Source: three-view drawing plus pictorial views. Frame: mm from the lowest corner of the part. Round coordinates to 2 decimals unless told otherwise and drop trailing zeros. Loops run counter-clockwise (first coordinate to the right, second up) from the corner with the lowest first, then second, coordinate; pieces in that order, holes last. Notation, with made-up numbers: (-39.75, 6.5) -> (16.25, 6.5) arc R14 cw to (16.25, 26.5) -> close; hole circle Ø9 at (-4.5, 33). An arc over 180 degrees is marked (long way). Answer in a Markdown table with one row per item. Add a question column.
Q1. Section C-C, the plane x = 54. Output: boundary loops of the cut face in (y, z), and give its area (3 significant figures).
Q2. Section D-D, the plane z = 42. Output: boundary loops of the cut face in (x, y), and give its area (3 significant figures).
Q3. Ray query, L1, parallel to Y at x = 71, z = 27; L2, parallel to X at y = 30, z = 50.5; L3, parallel to Z at x = 57, y = 38.5. Return the intervals inside material, ascending. Write a range as from..to.
Q4. Mould query, pull axis Z, two halves, no side actions, for the marked faces 1, 2 and 3. Classes: pulls with the +Z half, pulls with the -Z half, needs draft (parallel to the pull), parting line crosses it, or undercut.
Q5. Section A-A, the plane z = 27. Output: boundary loops of the cut face in (x, y), and give its area (3 significant figures).
Q6. Pin query (flat end, axial travel): pin 1 (3 mm diameter, centred on y = 48, z = 45.5, fed in from +X); pin 2 (3 mm diameter, centred on x = 49.5, y = 45.5, fed in from -Z); pin 3 (1 mm diameter, centred on x = 88.5, y = 17.5, fed in from +Z). Return the tip coordinate at first contact, or that it passes through.
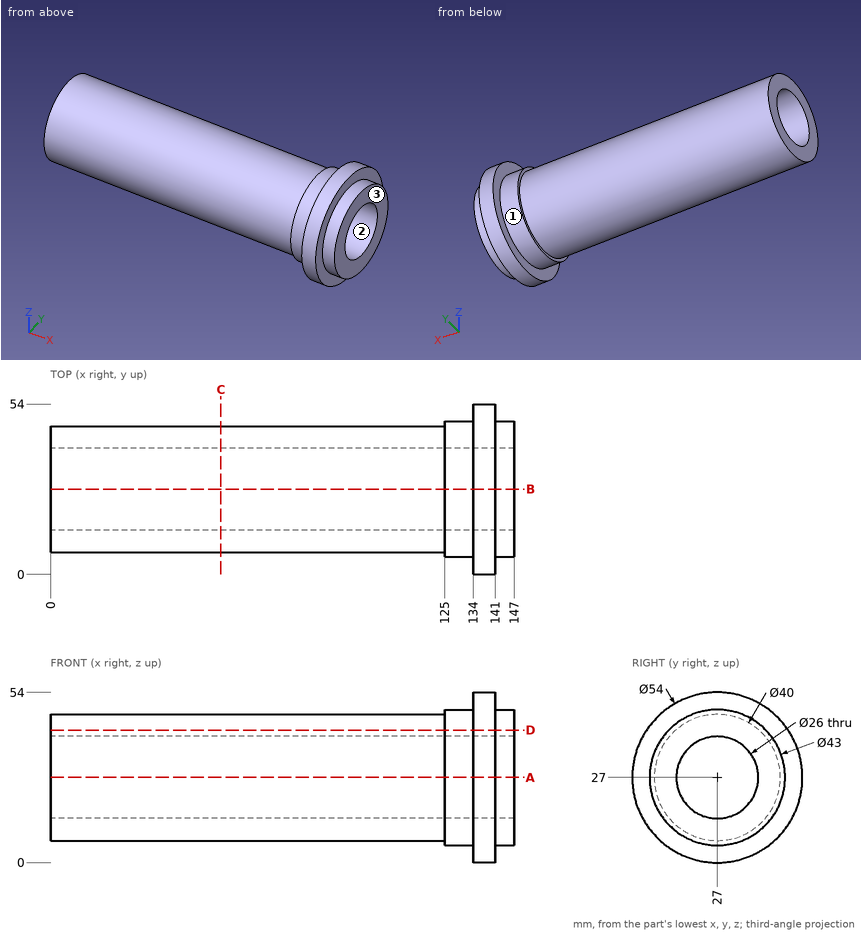
Answer block:
| question | item | result |
|---|---|---|
| 1 | outline | circle Ø40 at (27, 27); hole circle Ø26 at (27, 27) |
| 1 | area | 726 mm^2 |
| 2 | outline | (0, 13.77) -> (125, 13.77) -> (125, 11.6) -> (134, 11.6) -> (134, 4.55) -> (141, 4.55) -> (141, 11.6) -> (147, 11.6) -> (147, 42.4) -> (141, 42.4) -> (141, 49.45) -> (134, 49.45) -> (134, 42.4) -> (125, 42.4) -> (125, 40.23) -> (0, 40.23) -> close |
| 2 | area | 4,080 mm^2 |
| 3 | L1 | 7..14, 40..47 |
| 3 | L2 | 134..141 |
| 3 | L3 | 10.64..20.94, 33.06..43.36 |
| 4 | face 1 | parting line crosses it |
| 4 | face 2 | undercut |
| 4 | face 3 | needs draft |
| 5 | outline | (0, 7) -> (125, 7) -> (125, 5.5) -> (134, 5.5) -> (134, 0) -> (141, 0) -> (141, 5.5) -> (147, 5.5) -> (147, 14) -> (0, 14) -> close; (0, 40) -> (147, 40) -> (147, 48.5) -> (141, 48.5) -> (141, 54) -> (134, 54) -> (134, 48.5) -> (125, 48.5) -> (125, 47) -> (0, 47) -> close |
| 5 | area | 2,200 mm^2 |
| 6 | pin 1 | x = 141 |
| 6 | pin 2 | z = 16.46 |
| 6 | pin 3 | z = 44.86 |
